from build123d import *

# Parameters (mm, degrees)
SKETCH1_W           = 1000
SKETCH1_H           = 500
BOSS_EXTRUDE1_DEPTH = 35
M20_TAPPED_HOLE1_D  = 17.5
CHAMFER1_SIZE       = 15
CUT_EXTRUDE3_DEPTH  = 1130.97787589


with BuildPart() as part:
    # Sketch1 → Boss-Extrude1 (new body)
    with BuildSketch(Plane.XY):
        with Locations((-500, -275)):
            Rectangle(SKETCH1_W, SKETCH1_H)
    extrude(amount=-BOSS_EXTRUDE1_DEPTH)

    # M20 Tapped Hole1 (through all)
    with Locations(Plane(origin=(-30, -275, 0), x_dir=(1, 0, 0), z_dir=(0, 0, 1))):
        with Locations((0, 0), (-240, 0)):
            Hole(M20_TAPPED_HOLE1_D / 2)

    # Chamfer1
    chamfer1_edges = [part.edges().sort_by_distance(p)[0] for p in [
        (-500, -525, 0),
        (-500, -25, 0),
    ]]
    chamfer(chamfer1_edges, length=CHAMFER1_SIZE)

    # Sketch9 → Cut-Extrude3 (cut, through all)
    with BuildSketch(Plane.XY):
        Polygon((-500, 10), (0, 10), (0, -390), align=None)
    extrude(amount=-CUT_EXTRUDE3_DEPTH, mode=Mode.SUBTRACT)


solid = part.part
CAD build for the part. Positions are in the model's coordinates, mm. Coordinates: 2 decimals unless noted, no trailing zeros. Order: outer loops, then holes, each group sorted by start corner. A loop starts at its lowest first (then second) coordinate and runs counter-clockwise, first axis right, second up. Notation, with made-up numbers: (82, 32.25) -> (110, 32.25) arc R19 ccw to (110, 68.25) -> close; hole circle Ø10 at (40, 60). An arc over 180 degrees is marked (long way). Answer in a Markdown table with one row per item.
1) Band-saw the part on B-B (x = -109). List the corners of the cut face in (y, z).
Check values:
| item | result |
|---|---|
| outline | (-525, -35) -> (-302.8, -35) -> (-302.8, 0) -> (-510, 0) -> (-525, -15) -> close |
2) Mould opens along Y. For faces 1 (the face through (0, -458, -17)), 2 (the face through (-507, -525, -25)), 3 (the face through (-274.7, -267.62, -17.74)) say: pulls with the +Y half, pulls with the -Y half, needs draft (parallel to the pull), parting line crosses it, or undercut.
Check values:
| item | result |
|---|---|
| face 1 | needs draft |
| face 2 | pulls with the -Y half |
| face 3 | undercut |
3) Band-saw the part on D-D (x = -420.5). List the corners of the cut face in (y, z).
Check values:
| item | result |
|---|---|
| outline | (-525, -35) -> (-53.6, -35) -> (-53.6, 0) -> (-510, 0) -> (-525, -15) -> close |
4) Band-saw the part on C-C (y = -64). List the corners of the cut face in (x, z), and give its area (3 significant figures).
Check values:
| item | result |
|---|---|
| outline | (-1000, -35) -> (-407.5, -35) -> (-407.5, 0) -> (-1000, 0) -> close |
| area | 20,700 mm2 |
5) Flat gauge pins, fed straight in: P1, Ø1, axis at x = -156.5, z = -12.5, coming from the +Y side; P2, Ø1.5, axis at x = -344.5, z = -12.5, coming from the +Y side. Where does each tip first touch, or does it go through?
Check values:
| item | result |
|---|---|
| P1 | y = -264.4 |
| P2 | y = -113.8 |
6) Drill centre lines: line 1 (Y direction, x = -270, z = -17.5); line 2 (Y direction, x = -270, z = -13); line 3 (Y direction, x = -107, z = -30.5). Where is each one in solid material? Low to high.
Check values:
| item | result |
|---|---|
| line 1 | -525 to -283.75, -266.25 to -174 |
| line 2 | -523 to -283.75, -266.25 to -174 |
| line 3 | -525 to -304.4 |
7) Band-saw the part on A-A (z = -22). List the corners of the cut face in (x, y).
Check values:
| item | result |
|---|---|
| outline | (-1000, -525) -> (0, -525) -> (0, -390) -> (-456.25, -25) -> (-1000, -25) -> close; hole circle Ø17.5 at (-270, -275) |
